from build123d import *

# Parameters (mm, degrees)
EXTRUDE_1_DEPTH              = 17.5
HOLE_WIZARD_M4_1_D           = 3.3
HOLE_WIZARD_M4_1_DEPTH       = 9.5
HOLE_WIZARD_M4_1_TIP         = 0.991420021
HOLE_WIZARD_M6_1_D           = 5
HOLE_WIZARD_M6_1_DEPTH       = 12
HOLE_WIZARD_M6_1_CSINK_D     = 6.05
HOLE_WIZARD_M6_1_CSINK_ANGLE = 90
HOLE_WIZARD_M6_1_TIP         = 1.502151548


with BuildPart() as part:
    # 草图1 → 凸台-拉伸1 (new, symmetric)
    with BuildSketch(Plane.XY):
        with BuildLine():
            Line((-27.5, 27), (27.5, 27))
            Line((27.5, 27), (27.5, -17))
            Line((27.5, -17), (9, -17))
            Line((9, -17), (9, -13.228756555))
            ThreePointArc((9, -13.228756555), (0, 16), (-9, -13.228756555))
            Line((-9, -13.228756555), (-9, -17))
            Line((-9, -17), (-27.5, -17))
            Line((-27.5, -17), (-27.5, 27))
        make_face()
    extrude(amount=EXTRUDE_1_DEPTH, both=True)

    # M4 螺纹孔1
    with Locations(Plane.XY.offset(17.5)):
        with Locations((18.186533479, 10.5), (18.186533479, -10.5), (-18.186533479, -10.5), (-18.186533479, 10.5)):
            Hole(HOLE_WIZARD_M4_1_D / 2, depth=HOLE_WIZARD_M4_1_DEPTH)
            with Locations((0, 0, -(HOLE_WIZARD_M4_1_DEPTH + HOLE_WIZARD_M4_1_TIP / 2))):  # 118° drill point
                Cone(0, HOLE_WIZARD_M4_1_D / 2, HOLE_WIZARD_M4_1_TIP, mode=Mode.SUBTRACT)

    # M6 螺纹孔1
    with Locations(Plane(origin=(-20.5, 27, 10.5), x_dir=(0, 0, 1), z_dir=(0, 1, 0))):
        with Locations((0, 0), (-21, 0), (-21, 41), (0, 41)):
            CounterSinkHole(HOLE_WIZARD_M6_1_D / 2, HOLE_WIZARD_M6_1_CSINK_D / 2, depth=HOLE_WIZARD_M6_1_DEPTH, counter_sink_angle=HOLE_WIZARD_M6_1_CSINK_ANGLE)
            with Locations((0, 0, -(HOLE_WIZARD_M6_1_DEPTH + HOLE_WIZARD_M6_1_TIP / 2))):  # 118° drill point
                Cone(0, HOLE_WIZARD_M6_1_D / 2, HOLE_WIZARD_M6_1_TIP, mode=Mode.SUBTRACT)


solid = part.part
Work out the finished part from the listing and answer in its coordinate system (mm). A direction names the side the tool comes from. Round coordinates to 2 decimals unless told otherwise and drop trailing zeros. Write each loop counter-clockwise with the first axis right and the second up, starting at its lowest first coordinate (ties: lowest second). Pieces come first, ordered by that corner, then holes. Notation, with made-up numbers: (18.5, -39.75) -> (68.5, -39.75) arc R10 ccw to (68.5, -25.75) -> close; hole circle Ø7 at (47, 13). An arc over 180 degrees is marked (long way). Write each question's results on one line, items separated by ' | '.
Item 1: A cutting plane is placed at A-A, the plane y = -3.5. Determine the outline of the cut face in (x, z).
Result set:
outline: (-27.5, -17.5) -> (-15.61, -17.5) -> (-15.61, 17.5) -> (-27.5, 17.5) -> close; (15.61, -17.5) -> (27.5, -17.5) -> (27.5, 17.5) -> (15.61, 17.5) -> close
Item 2: The mould has two halves that part along X. Classify faces 6 (the face through (19.5, 9.5, 12.7)), 7 (the face through (6, 15, -17.5)): +X half, -X half, draft (parallel to the pull), parting line (faces both ways), or undercut.
Result set:
face 6: undercut | face 7: draft
Item 3: Flat-ended cylindrical pins translate along their axes: P1, Ø6, axis at x = -4.5, z = -12.5, coming from the -Y side; P2, Ø3, axis at x = 18.19, y = 10.5, coming from the +Z side; P3, Ø6.5, axis at x = -20.5, z = -10.5, coming from the +Y side. Find the tip coordinate at first contact, or state that the pin passes through.
Result set:
P1: y = 14.13 | P2: z = 7.91 | P3: y = 27
Item 4: A cutting plane is placed at D-D, the plane y = 21. Determine the outline of the cut face in (x, z), plus the area to 3 significant figures.
Result set:
outline: (-27.5, -17.5) -> (27.5, -17.5) -> (27.5, 17.5) -> (-27.5, 17.5) -> close; hole circle Ø5 at (-20.5, -10.5); hole circle Ø5 at (-20.5, 10.5); hole circle Ø5 at (20.5, -10.5); hole circle Ø5 at (20.5, 10.5) | area: 1,850 mm^2
Item 5: A cutting plane is placed at B-B, the plane x = -15. Determine the outline of the cut face in (y, z).
Result set:
outline: (-17, -17.5) -> (-5.57, -17.5) -> (-5.57, 17.5) -> (-17, 17.5) -> close; (5.57, -17.5) -> (27, -17.5) -> (27, 17.5) -> (5.57, 17.5) -> close
Item 6: A cutting plane is placed at C-C, the plane z = 15. Determine the outline of the cut face in (x, y).
Result set:
outline: (-27.5, -17) -> (-9, -17) -> (-9, -13.23) arc R16 cw (long way) to (9, -13.23) -> (9, -17) -> (27.5, -17) -> (27.5, 27) -> (-27.5, 27) -> close; hole circle Ø3.3 at (-18.19, -10.5); hole circle Ø3.3 at (-18.19, 10.5); hole circle Ø3.3 at (18.19, -10.5); hole circle Ø3.3 at (18.19, 10.5)
Item 7: Find the intervals of material crossed by line 1 along X through (y, z) = (-10, 15); line 2 along Z through (x, y) = (20, 14); line 3 along X through (y, z) = (0, 0.5), in increasing order. Write a range as [from, to].
Result set:
line 1: [-27.5, -19.76], [-16.61, -12.49], [12.49, 16.61], [19.76, 27.5] | line 2: [-17.5, -11.17], [-9.83, 9.83], [11.17, 17.5] | line 3: [-27.5, -16], [16, 27.5]
Item 8: Which of the six approach directions +Z, -Z, +X, -X, +Y, -Y give full straight-line access (tool end or side, diameter ignored) to faces 1 (the face through (9, -15, 0)), 2 (the face through (-18.02, 20.66, -10.17)), 3 (the face through (0, 27, 0)), 4 (the face through (-19.71, -11.13, 12.68)), 5 (the face through (6, 15, 17.5))?
Result set:
face 1: +Z, -Z, -Y | face 2: +Y | face 3: +Z, -Z, +X, -X, +Y | face 4: +Z | face 5: +Z, +X, -X, +Y, -Y
